from build123d import *

# Parameters (mm, degrees)
U_CHANNEL_DEPTH         = 55
FLANGE_PLATE_SKETCH_W   = 125.717283216
FLANGE_PLATE_SKETCH_H   = 164
FLANGE_PLATE_SKETCH_R   = 6
FLANGE_PLATE_DEPTH      = 5
CHANNEL_SIDE_TRIM_DEPTH = 171.979049299


with BuildPart() as part:
    # U-Channel Profile Sketch → U-Channel (new body)
    with BuildSketch(Plane.XY):
        with BuildLine():
            Line((35, 0), (35, 75))
            Line((35, 75), (30, 75))
            Line((30, 75), (30, 0))
            ThreePointArc((30, 0), (0, -30), (-30, 0))
            Line((-30, 0), (-30, 75))
            Line((-30, 75), (-35, 75))
            Line((-35, 75), (-35, 0))
            ThreePointArc((-35, 0), (0, -35), (35, 0))
        make_face()
    extrude(amount=U_CHANNEL_DEPTH)

    # Flange Plate Sketch → Flange Plate (add)
    with BuildSketch(Plane(origin=(0, 0, 0), x_dir=(-1, 0, 0), z_dir=(0, 0, -1))):
        with Locations((0.858641608, 20)):
            Rectangle(FLANGE_PLATE_SKETCH_W, FLANGE_PLATE_SKETCH_H)
        with Locations((48.717283216, -47)):
            Circle(FLANGE_PLATE_SKETCH_R, mode=Mode.SUBTRACT)
        with Locations((-47, -47)):
            Circle(FLANGE_PLATE_SKETCH_R, mode=Mode.SUBTRACT)
        with Locations((0, 87)):
            Circle(FLANGE_PLATE_SKETCH_R, mode=Mode.SUBTRACT)
    extrude(amount=-FLANGE_PLATE_DEPTH)

    # Channel Side Trim Sketch → Channel Side Trim (cut, through all)
    with BuildSketch(Plane(origin=(62, 0, 0), x_dir=(0, 0, -1), z_dir=(1, 0, 0))):
        Polygon((-55, 14), (-5, 75), (-55, 75), align=None)
    extrude(amount=-CHANNEL_SIDE_TRIM_DEPTH, mode=Mode.SUBTRACT)


solid = part.part
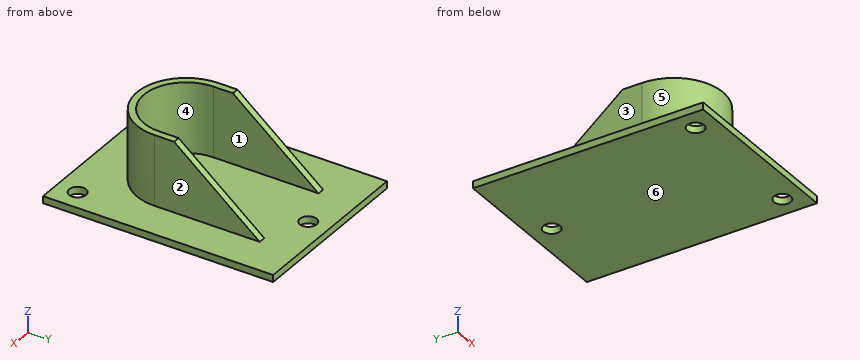
Can you work these out from the model? Positions are in its coordinate system, mm. Face numbers are marked on the shaded views. A direction names the side the tool comes from. Coordinates: 2 decimals unless noted, no trailing zeros. Order: outer loops, then holes, each group sorted by start corner. A loop starts at its lowest first (then second) coordinate and runs counter-clockwise, first axis right, second up. Notation, with made-up numbers: M 50.25,27 L 70.25,27 A19 cw 70.25,41 Z; hole C 64,-32 d4. An arc over 180 degrees is marked long. Write item = value, one per line.
(1) For the marked faces 1, 2 and 3, which set-ups out of +Z, -Z, +X, -X, +Y, -Y let a thin tool reach every point of the face, with its end or its side?
Results are:
face_1 = +Z, +Y
face_2 = +Z, +X, +Y, -Y
face_3 = +Z, -X, +Y, -Y
(2) I need wall thicknesses on line 1 along Y through (x, z) = (0, 3); line 2 along Y through (x, z) = (47, 1); line 3 along Z through (x, y) = (3.5, 47.5). Which ranges of each line are inside material? Lowest first, please. Write a range as [from, to].
Results are:
line_1 = [-62, 81], [93, 102]
line_2 = [-62, -53], [-41, 102]
line_3 = [0, 5]
(3) For pin 1 Ø3 at (x, y) = (-39, 46.5) entering from +Z; pin 2 Ø25 at (y, z) = (38.5, 34) entering from -X; pin 3 Ø15 at (y, z) = (50.5, 33) entering from +X, each with a flat end and sliding along its axis, tell me the tip position at first contact or that it passes through.
Results are:
pin_1 = 5
pin_2 = -35
pin_3 = 35
(4) Suppose I cut it at C-C on y = -47. Please give me the cut outline in (x, z).
Results are:
outline = M -63.72,0 L -54.72,0 L -54.72,5 L -63.72,5 Z; M -42.72,0 L 41,0 L 41,5 L -42.72,5 Z; M 53,0 L 62,0 L 62,5 L 53,5 Z
(5) Suppose I cut it at B-B on y = 87. Please give me the cut outline in (x, z).
Results are:
outline = M -63.72,0 L -6,0 L -6,5 L -63.72,5 Z; M 6,0 L 62,0 L 62,5 L 6,5 Z
(6) If we mould it in two halves opening along X, with no side actions, what happens to the marked faces 4, 5 and 6? For each: pulls with the +X half, pulls with the -X half, needs draft (parallel to the pull), parting line crosses it, or undercut.
Results are:
face_4 = undercut
face_5 = parting line crosses it
face_6 = needs draft
(7) Suppose I cut it at A-A on x = 0. Please give me the cut outline in (y, z).
Results are:
outline = M -62,0 L 81,0 L 81,5 L -30,5 L -30,55 L -35,55 L -35,5 L -62,5 Z; M 93,0 L 102,0 L 102,5 L 93,5 Z
(8) Suppose I cut it at D-D on z = 28. Please give me the cut outline in (x, y).
Results are:
outline = M -35,0 A35 ccw 35,0 L 35,46.94 L 30,46.94 L 30,0 A30 cw -30,0 L -30,46.94 L -35,46.94 Z
